CAD build for the part. Positions are in the model's coordinates, mm. A direction names the side the tool comes from. Give positions to 0.01 mm unless a question says otherwise; leave off trailing zeros. Loops run counter-clockwise (first coordinate to the right, second up) from the corner with the lowest first, then second, coordinate; pieces in that order, holes last.
```python
from build123d import *

# Parameters (mm, degrees)
SKETCH1_R                                           = 40
BOSS_EXTRUDE1_DEPTH                                 = 20
HOLE_SIZE_PER_SOCKET_HEAD_CAP_SCREW_TYP_D           = 11
HOLE_SIZE_PER_SOCKET_HEAD_CAP_SCREW_TYP_CBORE_D     = 18
HOLE_SIZE_PER_SOCKET_HEAD_CAP_SCREW_TYP_CBORE_DEPTH = 11


with BuildPart() as part:
    # Sketch1 → Boss-Extrude1 (new body)
    with BuildSketch(Plane(origin=(0, 0, 0), x_dir=(1, 0, 0), z_dir=(0, 1, 0))):
        with Locations(Location((0, 0, 0), (0, 0, 270))):
            Circle(SKETCH1_R)
    extrude(amount=BOSS_EXTRUDE1_DEPTH)

    # Hole size (per socket head cap screw type) 1 (through all)
    with Locations(Plane(origin=(-12.034248035, 20, 3.380365992), x_dir=(0, 0, 1), z_dir=(0, 1, 0))):
        with Locations((0, 0), (-6.760731984, 24.06849607)):
            CounterBoreHole(HOLE_SIZE_PER_SOCKET_HEAD_CAP_SCREW_TYP_D / 2, HOLE_SIZE_PER_SOCKET_HEAD_CAP_SCREW_TYP_CBORE_D / 2, HOLE_SIZE_PER_SOCKET_HEAD_CAP_SCREW_TYP_CBORE_DEPTH)


solid = part.part
```
1. Saw through at A-A, the plane x = -8. List the corners of the cut face in (y, z), and give its area (3 significant figures).
Responses:
outline: (0, -39.19) - (20, -39.19) - (20, -4.66) - (9, -4.66) - (9, -0.36) - (0, -0.36) - close; (0, 7.12) - (9, 7.12) - (9, 11.43) - (20, 11.43) - (20, 39.19) - (0, 39.19) - close
area: 1,320 mm2
2. Probe line 1 along Y through (x, z) = (13, -12); line 2 along Z through (x, y) = (-1, 1); line 3 along Z through (x, y) = (10.5, 18). List the from-to ranges inside material, lowest first.
Responses:
line 1: y = 0 to 9
line 2: z = -39.99 to 39.99
line 3: z = -38.6 to -12.25, 5.49 to 38.6
3. Saw through at D-D, the plane x = 13.5. List the corners of the cut face in (y, z), and give its area (3 significant figures).
Responses:
outline: (0, -37.65) - (20, -37.65) - (20, -12.26) - (9, -12.26) - (9, -8.68) - (0, -8.68) - close; (0, 1.92) - (9, 1.92) - (9, 5.5) - (20, 5.5) - (20, 37.65) - (0, 37.65) - close
area: 1,220 mm2
4. Saw through at B-B, the plane z = 0. List the corners of the cut face in (x, y), and give its area (3 significant figures).
Responses:
outline: (-40, 0) - (-16.37, 0) - (-16.37, 9) - (-20.38, 9) - (-20.38, 20) - (-40, 20) - close; (-7.7, 0) - (7.7, 0) - (7.7, 9) - (3.69, 9) - (3.69, 20) - (-3.69, 20) - (-3.69, 9) - (-7.7, 9) - close; (16.37, 0) - (40, 0) - (40, 20) - (20.38, 20) - (20.38, 9) - (16.37, 9) - close
area: 1,080 mm2
5. Tool access for faces 4 (the face through (6.665, 4.437, -2.188)), 5 (the face through (-20.82, 14.58, 1.43)): list every direction of +Z, -Z, +X, -X, +Y, -Y with a clear straight run to the whole face (end or side of a thin tool).
Responses:
face 4: +Y, -Y
face 5: +Y
6. Pull direction Z, two halves, no side cores. Call faces 1 (the face through (1, 20, -1)), 2 (the face through (-39.05, 9.86, -8.67)), 3 (the face through (6.558, 14.577, -10.522)): released by +Z, released by -Z, zero draft, split by the parting line, or undercut.
Responses:
face 1: zero draft
face 2: split by the parting line
face 3: undercut
7. Drop flat-ended pins along their axis: pin 1 (3 mm diameter, centred on x = -31.5, y = 10, fed in from -Z); pin 2 (3 mm diameter, centred on x = 29, y = 9, fed in from +Z); pin 3 (1.5 mm diameter, centred on x = 14.5, y = 15.5, fed in from -Z). Give the stop position or say it passes through.
Responses:
pin 1: stops at z = -26.46
pin 2: stops at z = 29.05
pin 3: stops at z = -37.56
8. Saw through at C-C, the plane y = 11. List the corners of the cut face in (x, z), and give its area (3 significant figures).
Responses:
outline: circle Ø80 at (0, 0); hole circle Ø18 at (-12.03, 3.38); hole circle Ø18 at (12.03, -3.38)
area: 4,520 mm2
